from build123d import *

# Parameters (mm, degrees)
BASE_PLATE_PROFILE_SKETCH_R = 8.363945013
BASE_PLATE_3_HOLE_DEPTH     = 10
BORED_LUG_PROFILE_SKETCH_R  = 10
BORED_LUG_DEPTH             = 8


with BuildPart() as part:
    # Base Plate Profile Sketch → Base Plate 3-Hole (new body)
    with BuildSketch(Plane(origin=(0, 0, 0), x_dir=(1, 0, 0), z_dir=(0, 1, 0))):
        with BuildLine():
            Line((68, 25), (68, -25))
            ThreePointArc((68, -25), (56.032896381, -41.958896227), (36.043982083, -36.367918187))
            ThreePointArc((36.043982083, -36.367918187), (19.637945422, -23.224109156), (-0.720723799, -17.985565246))
            ThreePointArc((-0.720723799, -17.985565246), (-18, 0), (-0.720723799, 17.985565246))
            ThreePointArc((-0.720723799, 17.985565246), (19.637945422, 23.224109156), (36.043982083, 36.367918187))
            ThreePointArc((36.043982083, 36.367918187), (56.032896381, 41.958896227), (68, 25))
        make_face()
        with Locations(Location((0, 0, 0), (0, 0, 270))):
            Circle(BASE_PLATE_PROFILE_SKETCH_R, mode=Mode.SUBTRACT)
        with Locations(Location((50, 25, 0), (0, 0, 270))):
            Circle(BASE_PLATE_PROFILE_SKETCH_R, mode=Mode.SUBTRACT)
        with Locations(Location((50, -25, 0), (0, 0, 90))):
            Circle(BASE_PLATE_PROFILE_SKETCH_R, mode=Mode.SUBTRACT)
    extrude(amount=BASE_PLATE_3_HOLE_DEPTH)

    # Bored Lug Profile Sketch → Bored Lug (add, symmetric)
    with BuildSketch(Plane.XY):
        with BuildLine():
            Line((68, 10), (53.71, 10))
            ThreePointArc((53.71, 10), (74.800840464, 21.756077977), (93.237910195, 37.347850827))
            ThreePointArc((93.237910195, 37.347850827), (129.268851943, 30.554159275), (109, 0))
            Line((109, 0), (68, 0))
            Line((68, 0), (68, 10))
        make_face()
        with Locations((109, 22)):
            Circle(BORED_LUG_PROFILE_SKETCH_R, mode=Mode.SUBTRACT)
    extrude(amount=BORED_LUG_DEPTH, both=True)


solid = part.part
Could you check a few things on this model? Use its own coordinates, in mm. A direction names the side the tool comes from. Coordinates: 2 decimals unless noted, no trailing zeros. Order: outer loops, then holes, each group sorted by start corner. A loop starts at its lowest first (then second) coordinate and runs counter-clockwise, first axis right, second up. Notation, with made-up numbers: (70, 9.25) -> (126, 9.25) arc R27 ccw to (126, 36.25) -> close; hole circle Ø9 at (57.5, -22.5). An arc over 180 degrees is marked (long way). One line per question, with ' | ' between items.
Q1. If I drill on L1, parallel to Z at x = 43, y = 8.5; L2, parallel to Y at x = 32.5, z = 3; L3, parallel to X at y = 5, z = -25, over which ranges is the centre line in solid material (lowest first)?
Return value:
L1: -41.58 to -29.58, -20.42 to 20.42, 29.58 to 41.58 | L2: 0 to 10 | L3: 22.88 to 41.64, 58.36 to 68
Q2. Imagine slicing it at D-D on x = 73. Please give me the cut outline in (y, z), and give its area (3 significant figures).
Return value:
outline: (0, -8) -> (20.53, -8) -> (20.53, 8) -> (0, 8) -> close | area: 329 mm²
Q3. I'm going to push flat-ended pins straight in: P1, Ø13, axis at x = 78, y = 13, coming from the -Z side; P2, Ø12, axis at x = 81, z = -12.5, coming from the +Y side; P3, Ø8, axis at y = 5.5, z = -16, coming from the +X side; P4, Ø21.5, axis at x = 50, z = -25, coming from the -Y side. Where does each tip first touch, or does it pass through?
Return value:
P1: z = -8 | P2: y = 29.59 | P3: x = 68 | P4: y = 0
Q4. Imagine slicing it at C-C on z = -27. Please give me the cut outline in (x, y), and give its area (3 significant figures).
Return value:
outline: (25.97, 0) -> (41.88, 0) -> (41.88, 10) -> (25.97, 10) -> close; (58.12, 0) -> (67.89, 0) -> (67.89, 10) -> (58.12, 10) -> close | area: 257 mm²
Q5. Imagine slicing it at B-B on y = 29.5. Please give me the cut outline in (x, z), and give its area (3 significant figures).
Return value:
outline: (84.86, -8) -> (102.39, -8) -> (102.39, 8) -> (84.86, 8) -> close; (115.61, -8) -> (129.68, -8) -> (129.68, 8) -> (115.61, 8) -> close | area: 505 mm²
Q6. Imagine slicing it at A-A on x = 50. Please give me the cut outline in (y, z), and give its area (3 significant figures).
Return value:
outline: (0, -43) -> (10, -43) -> (10, -33.36) -> (0, -33.36) -> close; (0, -16.64) -> (10, -16.64) -> (10, 16.64) -> (0, 16.64) -> close; (0, 33.36) -> (10, 33.36) -> (10, 43) -> (0, 43) -> close | area: 525 mm²
Q7. On a 3-axis mill with a long thin cutter (end or side, diameter ignored), from which of +Z, -Z, +X, -X, +Y, -Y can I reach the whole of each face in a straight line? I mean faces 5 (the face through (35, 10, -1)), 6 (the face through (32, 0, -1)), 7 (the face through (68, 5, -17)). Say none if no direction works.
Return value:
face 5: -X, +Y | face 6: +Z, -Z, +X, -X, -Y | face 7: -Z, +X, +Y, -Y
Q8. Thinking about a two-plate mould opening in Z: for faces 1 (the face through (41.707, 4.93, 26.089)), 2 (the face through (68, 5, 16)), 3 (the face through (56.324, 4.93, 41.853)), 4 (the face through (58.293, 4.93, -26.089)), which applies, pulls with the +Z half, pulls with the -Z half, needs draft (parallel to the pull), parting line crosses it, or undercut?
Return value:
face 1: undercut | face 2: needs draft | face 3: pulls with the +Z half | face 4: undercut
